Geometry: final body of the model. Coordinates: model frame, mm. A direction names the side the tool comes from. Give positions to 0.01 mm unless a question says otherwise; leave off trailing zeros. Write each loop counter-clockwise with the first axis right and the second up, starting at its lowest first coordinate (ties: lowest second). Pieces come first, ordered by that corner, then holes.
Q1. Pin query (flat end, axial travel): pin 1 Ø3 at (x, z) = (-16.5, -5) entering from +Y; pin 2 Ø6 at (y, z) = (-5.5, -0.5) entering from +X; pin 3 Ø6 at (x, y) = (-20.5, -1) entering from +Z; pin 4 Ø3 at (x, y) = (-97.5, 5) entering from -Z. Return the tip coordinate at first contact, or that it passes through.
Q2. Section B-B (x = -120). Return the cut outline in (y, z).
Q3. Section A-A (x = -15). Return the cut outline in (y, z), plus the area to 3 significant figures.
Q4. Line query: line 1 (Z direction, x = -36, y = 0.25); line 2 (X direction, y = 1.75, z = 6.75); line 3 (Z direction, x = -82.5, y = 0.25). Output: solid intervals per line, ascending.
Q5. Mould query, pull axis Z, two halves, no side actions, for faces 1 (the flat face through (-123, -4, -4)), 2 (the flat face through (-88, 5, 2.5)), 3 (the cylindrical face through (-10.114, -3.373, -2.15)). Classes: +Z half, -Z half, draft (parallel to the pull), parting line (faces both ways), or undercut.
Q6. Reachability of faces 4 (the cylindrical face through (-116.25, 5.02, 0.05)), 5 (the cylindrical face through (-36, 0, 5)), 6 (the cylindrical face through (-131, 0, 5)), 7 (the cylindrical face through (-129.54, -4.05, -2.58)) from +Z, -Z, +X, -X, +Y, -Y: full face, straight path, thin tool, end or side. Return the list, or none.
from build123d import *

# Parameters (mm, degrees)
CUT_EXTRUDE_START   = 4
CUT_EXTRUDE_1_DEPTH = 1.8
CHAMFER_1_SIZE      = 0.5
CUT_EXTRUDE_3_DEPTH = 3


with BuildPart() as part:
    # 草图1 → 旋转1 (revolve)
    with BuildSketch(Plane.XY, mode=Mode.PRIVATE) as revolve_1_sk:
        Polygon((-133, 5), (-130.1, 5), (-130.1, 4.8), (-129, 4.8), (-129, 5), (-123, 5), (-123, 6.5), (-54.5, 6.5), (-54.5, 8), (-51, 8), (-51, 5), (-20, 5), (-20, 4), (0, 4), (0, 0), (-133, 0), align=None)
    revolve(revolve_1_sk.sketch.rotate(Axis((0, 0, 0), (-1, 0, 0)), 90), axis=Axis((0, 0, 0), (-1, 0, 0)))

    # 草图2 → 切除-拉伸1 (cut)
    with BuildSketch(Plane(origin=(0, 0, 0), x_dir=(1, 0, 0), z_dir=(0, 1, 0)).offset(CUT_EXTRUDE_START)):
        with BuildLine():
            Line((-10, 1.5), (0, 1.5))
            ThreePointArc((0, 1.5), (1.5, 0), (0, -1.5))
            Line((0, -1.5), (-10, -1.5))
            ThreePointArc((-10, -1.5), (-11.5, 0), (-10, 1.5))
        make_face()
    extrude(amount=-CUT_EXTRUDE_1_DEPTH, mode=Mode.SUBTRACT)

    # 倒角1
    chamfer_1_edges = [part.edges().sort_by_distance(p)[0] for p in [
        (-20, 0, 5),
        (-51, 0, 8),
        (-123, 0, 6.5),
        (-133, 0, 5),
        (0, -3.31662479, 2.236067977),
    ]]
    chamfer(chamfer_1_edges, length=CHAMFER_1_SIZE)

    # 草图4 → 切除-拉伸3 (cut)
    with BuildSketch(Plane(origin=(0, 6.5, 0), x_dir=(1, 0, 0), z_dir=(0, 1, 0))):
        with BuildLine():
            Line((-113.75, 2.5), (-63.75, 2.5))
            ThreePointArc((-63.75, 2.5), (-61.25, 0), (-63.75, -2.5))
            Line((-63.75, -2.5), (-113.75, -2.5))
            ThreePointArc((-113.75, -2.5), (-116.25, 0), (-113.75, 2.5))
        make_face()
    extrude(amount=-CUT_EXTRUDE_3_DEPTH, mode=Mode.SUBTRACT)


solid = part.part
Computed:
1. pin 1: stops at y = 1.94
1. pin 2: stops at x = 0
1. pin 3: stops at z = 5
1. pin 4: stops at z = -5.48
2. outline: circle Ø13 at (0, 0)
3. outline: circle Ø8 at (0, 0)
3. area: 50.3 mm2
4. line 1: z = -4.99 to 4.99
4. line 2: x = -54.5 to -51
4. line 3: z = -6.5 to 6.5
5. face 1: draft
5. face 2: undercut
5. face 3: parting line
6. face 4: +Y
6. face 5: +X
6. face 6: -X
6. face 7: none
